from build123d import *

# Parameters (mm, degrees)
SKETCH1_R               = 5.9
BOSS_EXTRUDE1_DEPTH     = 35.4
M4_TAPPED_HOLE1_D       = 3.3
M4_TAPPED_HOLE1_DEPTH   = 10.1
M4_TAPPED_HOLE1_TIP     = 0.991420021
SKETCH5_R               = 6
SKETCH5_R_2             = 4
BOSS_EXTRUDE2_DEPTH     = 20
CHAMFER1_SIZE           = 1
CUT_EXTRUDE1_DEPTH      = 37.402747149
CUT_EXTRUDE1_DEPTH_BACK = 37.402747149
SKETCH6_W               = 2.026292368
SKETCH6_H               = 10
SKETCH7_OUTSIDE_W       = 22.93
SKETCH7_OUTSIDE_H       = 22.93
CUT_EXTRUDE2_DEPTH      = 23.927930565


with BuildPart() as part:
    # Sketch1 → Boss-Extrude1 (new body)
    with BuildSketch(Plane.XY):
        Circle(SKETCH1_R)
    extrude(amount=BOSS_EXTRUDE1_DEPTH)

    # Sketch2 → Revolve1 (revolve)
    with BuildSketch(Plane(origin=(0, 0, 0), x_dir=(1, 0, 0), z_dir=(0, 1, 0))):
        with BuildLine():
            Line((0, 5.9), (0, 0))
            Line((0, 0), (-5.9, 0))
            ThreePointArc((-5.9, 0), (-4.171930009, 4.171930009), (0, 5.9))
        make_face()
    revolve(axis=Axis((0, 0, -5.9), (0, 0, 1)))

    # M4 Tapped Hole1
    with Locations(Plane.XY.offset(35.4)):
        with Locations((0, 0)):
            Hole(M4_TAPPED_HOLE1_D / 2, depth=M4_TAPPED_HOLE1_DEPTH)
            with Locations((0, 0, -(M4_TAPPED_HOLE1_DEPTH + M4_TAPPED_HOLE1_TIP / 2))):  # 118° drill point
                Cone(0, M4_TAPPED_HOLE1_D / 2, M4_TAPPED_HOLE1_TIP, mode=Mode.SUBTRACT)

    # Sketch5 → Boss-Extrude2 (add)
    with BuildSketch(Plane.XY.offset(35.4)):
        Circle(SKETCH5_R)
        Circle(SKETCH5_R_2, mode=Mode.SUBTRACT)
    extrude(amount=-BOSS_EXTRUDE2_DEPTH)

    # Chamfer1
    chamfer1_edges = [part.edges().sort_by_distance(p)[0] for p in [
        (-6, 0, 35.4),
    ]]
    chamfer(chamfer1_edges, length=CHAMFER1_SIZE)

    # Sketch6 → Cut-Extrude1 (cut, two sides: drawn at the far end of the back side and taken through both)
    with BuildSketch(Plane(origin=(0, 0, 0), x_dir=(1, 0, 0), z_dir=(0, 1, 0)).offset(-CUT_EXTRUDE1_DEPTH_BACK)):
        with Locations((-6.513146184, -24.4)):
            Rectangle(SKETCH6_W, SKETCH6_H)
        with Locations((6.513146184, -24.4)):
            Rectangle(SKETCH6_W, SKETCH6_H)
    extrude(amount=CUT_EXTRUDE1_DEPTH + CUT_EXTRUDE1_DEPTH_BACK, mode=Mode.SUBTRACT)

    # Sketch7 outside → Cut-Extrude2 (cut, through all)
    with BuildSketch(Plane(origin=(0, 0, 15.4), x_dir=(-1, 0, 0), z_dir=(0, 0, -1))):
        Rectangle(SKETCH7_OUTSIDE_W, SKETCH7_OUTSIDE_H)
        with BuildLine():
            Line((-1.25, 5.766064516), (-4.5790389, 0))
            Line((-4.5790389, 0), (-1.25, -5.766064516))
            ThreePointArc((-1.25, -5.766064516), (0, -5.9), (1.25, -5.766064516))
            Line((1.25, -5.766064516), (4.5790389, 0))
            Line((4.5790389, 0), (1.25, 5.766064516))
            ThreePointArc((1.25, 5.766064516), (0, 5.9), (-1.25, 5.766064516))
        make_face(mode=Mode.SUBTRACT)
    extrude(amount=CUT_EXTRUDE2_DEPTH, mode=Mode.SUBTRACT)


solid = part.part
Can you work these out from the model? Positions are in its coordinate system, mm. A direction names the side the tool comes from. Coordinates: 2 decimals unless noted, no trailing zeros. Write each loop counter-clockwise with the first axis right and the second up, starting at its lowest first coordinate (ties: lowest second). Pieces come first, ordered by that corner, then holes. Notation, with made-up numbers: M -14,53 L -9,53 A19 cw -9,83 Z; hole C 57.25,-14.5 d11. An arc over 180 degrees is marked long. Use one line per item in the form item = value.
Q1. We'd pull the mould along Y, two halves only. Please class faces 5 (the cylindrical face through (-4.76, -3.65, 25.03)), 6 (the flat face through (2.891, 2.923, 5.654)), 7 (the cylindrical face through (1.216, 1.115, 30.279)): +Y half, -Y half, draft (parallel to the pull), parting line (faces both ways), or undercut.
Model answer:
face_5 = parting line
face_6 = +Y half
face_7 = undercut
Q2. If we section it at B-B (z = 22): Write out the boundary of the cut face in (x, y), then the cut area to 3 significant figures.
Model answer:
outline = M -5.5,-2.4 A6 ccw 5.5,-2.4 L 5.5,2.4 A6 ccw -5.5,2.4 Z
area = 110 mm^2
Q3. For faces 1 (the flat face through (2.94, -2.84, 5.65)), 2 (the flat face through (-2.891, -2.923, 5.654)), 3 (the flat face through (-4, 2, 15.4)), 4 (the flat face through (5.5, 0, 24)), which set-ups out of +Z, -Z, +X, -X, +Y, -Y let a thin tool reach every point of the face, with its end or its side?
Model answer:
face_1 = -Z, +X, -Y
face_2 = -Z, -X, -Y
face_3 = -Z
face_4 = +X, +Y, -Y
Q4. For P1, Ø2, axis at y = -3.5, z = 29, coming from the +X side; P2, Ø2, axis at x = -3.5, z = 13.5, coming from the -Y side; P3, Ø2.5, axis at y = 0, z = 24.5, coming from the -X side, each with a flat end and sliding along its axis, tell me the tip position at first contact or that it passes through.
Model answer:
P1 = 5.45
P2 = -3.6
P3 = -5.5
Q5. If we section it at A-A (z = 15): Write out the boundary of the cut face in (x, y).
Model answer:
outline = M -4.58,0 L -1.25,-5.77 A5.9 ccw 1.25,-5.77 L 4.58,0 L 1.25,5.77 A5.9 ccw -1.25,5.77 Z
Q6. I need wall thicknesses on line 1 along X through (y, z) = (0, 29); line 2 along Y through (x, z) = (0, 28.75). Which ranges of each line are inside material? Lowest first, please. Write a range as from..to.
Model answer:
line_1 = -5.5..-1.65, 1.65..5.5
line_2 = -6..-1.65, 1.65..6
